```python
from build123d import *

# Parameters (mm, degrees)
EXTRUDE_671_DEPTH        = 1730
SKETCH_2_W               = 49
SKETCH_2_H               = 55.5
EXTRUDE_1_DEPTH          = 85
SKETCH_4_W               = 49
SKETCH_4_H               = 55.5
EXTRUDE_3_DEPTH          = 95
SKETCH_9_R               = 23.5
CUT_EXTRUDE_5_DEPTH      = 3
SKETCH_10_R              = 6
EXTRUDE_4_DEPTH          = 28
CHAMFER_1_SIZE           = 1
PATTERN_CIRCULAR_1_COUNT = 4


with BuildPart() as part:
    # 草图1 → Extrude 671 (new body)
    with BuildSketch(Plane.XY):
        Polygon((15, 50), (15, 43), (35, 43), (35, 50), (50, 50), (50, 20), (42, 20), (42, 10), (50, 10), (50, 0), (0, 0), (0, 10), (8, 10), (8, 20), (0, 20), (0, 50), align=None)
    extrude(amount=EXTRUDE_671_DEPTH)

    # 草图2 → 凸台-拉伸1 (add)
    with BuildSketch(Plane.XY.offset(1730)):
        with Locations((25, 27.75)):
            Rectangle(SKETCH_2_W, SKETCH_2_H)
    extrude(amount=EXTRUDE_1_DEPTH)

    # 草图4 → 凸台-拉伸3 (add)
    with BuildSketch(Plane(origin=(0, 0, 0), x_dir=(-1, 0, 0), z_dir=(0, 0, -1))):
        with Locations((-25, 27.75)):
            Rectangle(SKETCH_4_W, SKETCH_4_H)
    extrude(amount=EXTRUDE_3_DEPTH)

    # 草图9 → 切除-拉伸5 (cut)
    with BuildSketch(Plane(origin=(49.5, 0, 0), x_dir=(0, 0, -1), z_dir=(1, 0, 0))):
        with Locations((56, 27.75)):
            Circle(SKETCH_9_R)
    cut_extrude_5 = extrude(amount=-CUT_EXTRUDE_5_DEPTH, mode=Mode.SUBTRACT)

    # 草图10 → 凸台-拉伸4 (add)
    with BuildSketch(Plane(origin=(46.5, 0, 0), x_dir=(0, 0, -1), z_dir=(1, 0, 0))):
        with Locations((56, 27.75)):
            Circle(SKETCH_10_R)
    extrude_4 = extrude(amount=EXTRUDE_4_DEPTH)

    # 倒角1
    chamfer_1_edges = [part.edges().sort_by_distance(p)[0] for p in [
        (74.5, 27.75, -50),
    ]]
    chamfer(chamfer_1_edges, length=CHAMFER_1_SIZE)

    # 草图12 → M5 螺纹孔1 (revolve, cut)
    with BuildSketch(Plane(origin=(50, 47.75, -76), x_dir=(0, 0, -1), z_dir=(0, 1, 0))):
        Polygon((0, 0), (0, 15.2618073), (2.1, 14), (2.1, 10), (2.5, 10), (2.5, 0), align=None)
    hole_wizard_m5_1 = revolve(axis=Axis((56.35, 47.75, -76), (-1, 0, 0)), mode=Mode.SUBTRACT)

    # 阵列(圆周)1: M5 螺纹孔1 ×4 about axis
    pattern_circular_1_axis = Axis((0, 27.75, -56), (1, 0, 0))
    for i in range(1, PATTERN_CIRCULAR_1_COUNT):
        add(hole_wizard_m5_1.rotate(pattern_circular_1_axis, i * 360 / PATTERN_CIRCULAR_1_COUNT), mode=Mode.SUBTRACT)

    # 镜向1: 切除-拉伸5, 凸台-拉伸4, M5 螺纹孔1 across plane
    add(cut_extrude_5.mirror(Plane(origin=(25, 0, 0), x_dir=(0, 0, 1), z_dir=(1, 0, 0))), mode=Mode.SUBTRACT)
    add(extrude_4.mirror(Plane(origin=(25, 0, 0), x_dir=(0, 0, 1), z_dir=(1, 0, 0))))
    add(hole_wizard_m5_1.mirror(Plane(origin=(25, 0, 0), x_dir=(0, 0, 1), z_dir=(1, 0, 0))), mode=Mode.SUBTRACT)

    # 镜向1 copy 1 sketch → 镜向1 copy 1 (revolve, cut)
    with BuildSketch(Plane(origin=(0, 47.75, -36), x_dir=(0, 1, 0), z_dir=(0, 0, 1))):
        Polygon((0, 0), (0, -15.2618073), (2.1, -14), (2.1, -10), (2.5, -10), (2.5, 0), align=None)
    revolve(axis=Axis((-6.35, 47.75, -36), (-1, 0, 0)), mode=Mode.SUBTRACT)

    # 镜向1 copy 2 sketch → 镜向1 copy 2 (revolve, cut)
    with BuildSketch(Plane(origin=(0, 7.75, -36), x_dir=(0, 0, 1), z_dir=(0, -1, 0))):
        Polygon((0, 0), (0, -15.2618073), (2.1, -14), (2.1, -10), (2.5, -10), (2.5, 0), align=None)
    revolve(axis=Axis((-6.35, 7.75, -36), (-1, 0, 0)), mode=Mode.SUBTRACT)

    # 镜向1 copy 3 sketch → 镜向1 copy 3 (revolve, cut)
    with BuildSketch(Plane(origin=(0, 7.75, -76), x_dir=(0, -1, 0), z_dir=(0, 0, -1))):
        Polygon((0, 0), (0, -15.2618073), (2.1, -14), (2.1, -10), (2.5, -10), (2.5, 0), align=None)
    revolve(axis=Axis((-6.35, 7.75, -76), (-1, 0, 0)), mode=Mode.SUBTRACT)


solid = part.part
```
Geometry: final body of the model. Coordinates: model frame, mm. A direction names the side the tool comes from. Round coordinates to 2 decimals unless told otherwise and drop trailing zeros. Order: outer loops, then holes, each group sorted by start corner. A loop starts at its lowest first (then second) coordinate and runs counter-clockwise, first axis right, second up. Notation, with made-up numbers: (-36, 27.5) - (21, 27.5) arc R15 ccw to (21, 49.5) - close; hole circle Ø3 at (-6.5, 14.25). An arc over 180 degrees is marked (long way). Use CSV: the item, a comma, the result in double quotes. Start each with the question number.
Q1. Material intervals for line 1 along Z through (x, y) = (45, 47); line 2 along Y through (x, z) = (38, -36); line 3 along Z through (x, y) = (3, 27.5), sorted ascending. Write a range as from..to.
Q2. Section query A-A (z = 146.5). Return loops of the section in (x, y).
Q3. Access query for faces 1 (the face through (50, 35, 853)), 2 (the face through (3.5, 23, -61)), 3 (the face through (46.5, 23, -61)). Directions: +Z, -Z, +X, -X, +Y, -Y. A direction counts if a zero-diameter tool reaches every point of the face in a straight line with its end or side. Return the directions, or none.
Q4. Mould query, pull axis Y, two halves, no side actions, for faces 4 (the face through (1.98, 13.45, -37.35)), 5 (the face through (25, 55.5, 1772)), 6 (the face through (0, 35, 853)). Classes: +Y half, -Y half, draft (parallel to the pull), parting line (faces both ways), or undercut.
Q5. First-contact query: pin 1 (6 mm diameter, centred on x = 49, z = 356, fed in from -Y); pin 2 (6 mm diameter, centred on y = 17.5, z = 1174.5, fed in from +X); pin 3 (4.5 mm diameter, centred on x = 10.5, z = 1003.5, fed in from +Y); pin 4 (6.5 mm diameter, centred on y = 47.75, z = -76, fed in from +X). Flat tips, straight axial feed; report the tip coordinate or a pass-through.
Result set:
1,line 1,"z = -95..-78.38, -73.62..-38.38, -33.62..1815"
1,line 2,"y = 0..5.65, 9.85..45.65, 49.85..55.5"
1,line 3,"z = -95..-79.5, -61.99..-50.01, -32.5..1815"
2,outline,"(0, 0) - (50, 0) - (50, 10) - (42, 10) - (42, 20) - (50, 20) - (50, 50) - (35, 50) - (35, 43) - (15, 43) - (15, 50) - (0, 50) - (0, 20) - (8, 20) - (8, 10) - (0, 10) - close"
3,face 1,"+Z, +X, +Y, -Y"
3,face 2,"-X"
3,face 3,"+X"
4,face 4,"undercut"
4,face 5,"+Y half"
4,face 6,"draft"
5,pin 1,"stops at y = 0"
5,pin 2,"stops at x = 50"
5,pin 3,"stops at y = 50"
5,pin 4,"stops at x = 49.5"
